Here's how the part is built. I have some questions about the finished solid (model axes, mm). A direction names the side the tool comes from. Give positions to 0.01 mm unless a question says otherwise; leave off trailing zeros. Loops run counter-clockwise (first coordinate to the right, second up) from the corner with the lowest first, then second, coordinate; pieces in that order, holes last.
Q1. For faces 1 (the face through (2, 0.1, 7.5)), 2 (the face through (10.44, 10.74, -2.38)), 3 (the face through (17, 8, 7)), 4 (the face through (2, -4, 0)), which set-ups out of +Z, -Z, +X, -X, +Y, -Y let a thin tool reach every point of the face, with its end or its side?
Q2. Suppose I cut it at D-D (x = 1.75). List the corners of the cut face in (y, z) for me.
Q3. I need wall thicknesses on probe 1 along Z at (x, y) = (16.25, -7.5); probe 2 along X at (y, z) = (-10, 4.5); probe 3 along X at (y, z) = (-11, -1.25). Which ranges of each line are inside material? Lowest first, please.
Q4. Suppose I cut it at B-B (y = 0). List the corners of the cut face in (x, z) for me.
Q5. Suppose I cut it at C-C (x = 13.25). List the corners of the cut face in (y, z) for me, and give its area (3 significant figures).
Q6. Suppose I cut it at A-A (z = 0). List the corners of the cut face in (x, y) for me, and give its area (3 significant figures).
Q7. I'm going to push flat-ended pins straight in: P1, Ø1, axis at y = 2, z = 0.5, coming from the +X side; P2, Ø1, axis at y = -2.5, z = -4.5, coming from the +X side; P3, Ø1.5, axis at x = 5, y = 2, coming from the -Z side. Where does each tip first touch, or does it pass through?
```python
from build123d import *

# Parameters (mm, degrees)
CHAMFER1_SIZE       = 1
SKETCH5_OUTSIDE_W   = 34.778
SKETCH5_OUTSIDE_H   = 34.778
SKETCH5_OUTSIDE_W_2 = 16.801740482
SKETCH5_OUTSIDE_H_2 = 8
CUT_EXTRUDE2_DEPTH  = 4
CUT_EXTRUDE3_START  = -3
SKETCH7_R           = 10.1
SKETCH7_R_2         = 10
CUT_EXTRUDE3_DEPTH  = 3


with BuildPart() as part:
    # Sketch1 → Revolve1 (revolve)
    with BuildSketch(Plane(origin=(0, 0, 0), x_dir=(1, 0, 0), z_dir=(0, 1, 0)), mode=Mode.PRIVATE) as revolve1_sk:
        Polygon((0, 0), (17, 0), (17, 12.4), (15, 12.4), (15, 11), (6, 11), (6, 10), (4, 10), (4, 7.5), (0, 7.5), align=None)
    revolve(revolve1_sk.sketch.rotate(Axis((0, 0, 0), (1, 0, 0)), 180), axis=Axis((0, 0, 0), (1, 0, 0)))

    # Sketch3 → Revolve2 (revolve)
    with BuildSketch(Plane.XY):
        with BuildLine():
            Line((9, 0), (9, 10))
            Line((9, 10), (17, 10))
            ThreePointArc((17, 10), (18.495097568, 5.099019514), (19, 0))
            Line((19, 0), (9, 0))
        make_face()
    revolve(axis=Axis((9, 0, 0), (1, 0, 0)))

    # Chamfer1
    chamfer1_edges = [part.edges().sort_by_distance(p)[0] for p in [
        (17, 0, -12.4),
    ]]
    chamfer(chamfer1_edges, length=CHAMFER1_SIZE)

    # Sketch5 outside → Cut-Extrude2 (cut)
    with BuildSketch(Plane.ZY):
        Rectangle(SKETCH5_OUTSIDE_W, SKETCH5_OUTSIDE_H)
        Rectangle(SKETCH5_OUTSIDE_W_2, SKETCH5_OUTSIDE_H_2, mode=Mode.SUBTRACT)
    extrude(amount=-CUT_EXTRUDE2_DEPTH, mode=Mode.SUBTRACT)

    # Sketch7 → Cut-Extrude3 (cut)
    with BuildSketch(Plane(origin=(17, 0, 0), x_dir=(0, 0, -1), z_dir=(1, 0, 0)).offset(CUT_EXTRUDE3_START)):
        Circle(SKETCH7_R)
        with Locations(Location((0, 0, 0), (0, 0, 180))):
            Circle(SKETCH7_R_2, mode=Mode.SUBTRACT)
    extrude(amount=CUT_EXTRUDE3_DEPTH, mode=Mode.SUBTRACT)


solid = part.part
```
Solutions:
1. face 1: +Z, -X
1. face 2: -X
1. face 3: +X
1. face 4: +Z, -Z, -X, -Y
2. outline: (-4, -6.34) arc R7.5 ccw to (4, -6.34) - (4, 6.34) arc R7.5 ccw to (-4, 6.34) - close
3. probe 1: z = -9.56 to -6.76, -6.61 to 6.61, 6.76 to 9.56
3. probe 2: x = 6 to 17
3. probe 3: x = 15 to 17
4. outline: (0, -7.5) - (4, -7.5) - (4, -10) - (6, -10) - (6, -11) - (15, -11) - (15, -12.4) - (16, -12.4) - (17, -11.4) - (17, -10.1) - (14, -10.1) - (14, -10) - (17, -10) arc R26 ccw to (17, 10) - (14, 10) - (14, 10.1) - (17, 10.1) - (17, 11.4) - (16, 12.4) - (15, 12.4) - (15, 11) - (6, 11) - (6, 10) - (4, 10) - (4, 7.5) - (0, 7.5) - close
5. outline: circle Ø22 at (0, 0)
5. area: 380 mm2
6. outline: (0, -4) - (4, -4) - (4, -10) - (6, -10) - (6, -11) - (15, -11) - (15, -12.4) - (16, -12.4) - (17, -11.4) - (17, -10.1) - (14, -10.1) - (14, -10) - (17, -10) arc R26 ccw to (17, 10) - (14, 10) - (14, 10.1) - (17, 10.1) - (17, 11.4) - (16, 12.4) - (15, 12.4) - (15, 11) - (6, 11) - (6, 10) - (4, 10) - (4, 4) - (0, 4) - close
6. area: 345 mm2
7. P1: stops at x = 18.95
7. P2: stops at x = 18.58
7. P3: stops at z = -9.92
